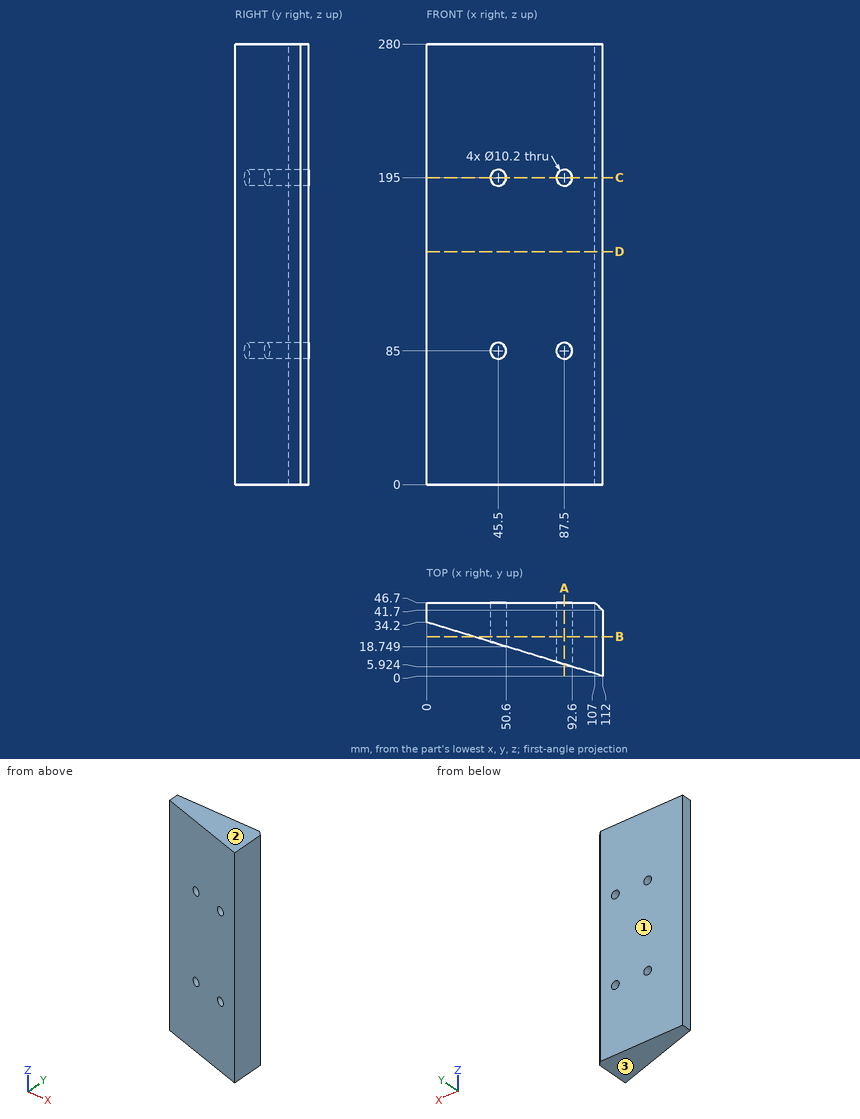
Print and shaded views of the part. All mm, measured from the part's lowest x, y and z. Coordinates: 2 decimals unless noted, no trailing zeros. Order: outer loops, then holes, each group sorted by start corner. A loop starts at its lowest first (then second) coordinate and runs counter-clockwise, first axis right, second up. Notation, with made-up numbers: M -19.75,-16 L -7.75,-16 A18 ccw -7.75,12 Z; hole C 70.5,-2 d5. An arc over 180 degrees is marked long. Answer as CSV lines item,"result".
1) Drill centre lines: L1, parallel to Z at x = 45.5, y = 38.5; L2, parallel to X at y = 20, z = 195; L3, parallel to Y at x = 106, z = 182. Where is each one in solid material? Low to high. Write a range as from..to.
Verdict:
L1,"0..79.9, 90.1..189.9, 200.1..280"
L2,"50.6..82.4, 92.6..112"
L3,"1.83..46.7"
2) Cut at A-A (x = 87.5). List the corners of the cut face in (y, z).
Verdict:
outline,"M 7.48,0 L 46.7,0 L 46.7,79.9 L 7.48,79.9 Z; M 7.48,90.1 L 46.7,90.1 L 46.7,189.9 L 7.48,189.9 Z; M 7.48,200.1 L 46.7,200.1 L 46.7,280 L 7.48,280 Z"
3) Mould opens along Z. For the marked faces 1, 2 and 3 say: released by +Z, released by -Z, zero draft, split by the parting line, or undercut.
Verdict:
face 1,"zero draft"
face 2,"released by +Z"
face 3,"released by -Z"
4) Flat gauge pins, fed straight in: P1, Ø6, axis at x = 45.5, z = 195, coming from the -Y side; P2, Ø11.5, axis at x = 45.5, z = 85, coming from the -Y side; P3, Ø5, axis at x = 17.5, z = 205.5, coming from the -Y side; P4, Ø5, axis at x = 54.5, z = 186.5, coming from the -Y side. Where does each tip first touch, or does it go through?
Verdict:
P1,"through"
P2,"y = 18.55"
P3,"y = 28.09"
P4,"y = 16.79"
5) Cut at B-B (y = 25). List the corners of the cut face in (x, z).
Verdict:
outline,"M 30.13,0 L 112,0 L 112,280 L 30.13,280 Z; hole C 45.5,85 d10.2; hole C 45.5,195 d10.2; hole C 87.5,85 d10.2; hole C 87.5,195 d10.2"
6) Cut at C-C (z = 195). List the corners of the cut face in (x, y), then the cut area to 3 significant figures.
Verdict:
outline,"M 0,34.2 L 40.4,21.86 L 40.4,46.7 L 0,46.7 Z; M 50.6,18.75 L 82.4,9.04 L 82.4,46.7 L 50.6,46.7 Z; M 92.6,5.92 L 112,0 L 112,41.7 L 107,46.7 L 92.6,46.7 Z"
area,"2,630 mm2"
7) Cut at D-D (z = 148). List the corners of the cut face in (x, y).
Verdict:
outline,"M 0,34.2 L 112,0 L 112,41.7 L 107,46.7 L 0,46.7 Z"
